Verification items for the finished model (mm, model axes). A direction names the side the tool comes from. Coordinates: 2 decimals unless noted, no trailing zeros. Order: outer loops, then holes, each group sorted by start corner. A loop starts at its lowest first (then second) coordinate and runs counter-clockwise, first axis right, second up.
Q1. Thickness scan on line 1 (Y direction, x = 0.7, z = 1.4); line 2 (X direction, y = 4.9, z = -1.35); line 3 (X direction, y = 2.65, z = 0.5). Record the ranges inside material, lowest first.
Q2. Cross-section at A-A, the plane x = 0. Record the boundary of the cut face in (y, z).
Q3. Cross-section at C-C, the plane y = 3.75. Record the boundary of the cut face in (x, z).
Q4. Cross-section at D-D, the plane y = 2.6. Record the boundary of the cut face in (x, z), and give its area (3 significant figures).
Q5. Cross-section at B-B, the plane z = 0. Record the boundary of the cut face in (x, y), and give its area (3 significant figures).
Q6. Set-up check for faces 1 (the flat face through (0, 0, 0)), 2 (the cylindrical face through (0.45, 1.58, 1.43)): record each of +Z, -Z, +X, -X, +Y, -Y from which the full face is reachable in a straight line by a thin tool's end or side.
Q7. Depth check by flat-ended pin: P1, Ø2, axis at y = 1, z = 1.5, coming from the +X side; P2, Ø1, axis at y = 3.5, z = 1, coming from the -X side. Enter the tip coordinate at first touch or a pass-through.
from build123d import *

# Parameters (mm, degrees)
SKETCH1_R           = 1.5
BOSS_EXTRUDE1_DEPTH = 3
SKETCH2_R           = 2
BOSS_EXTRUDE2_DEPTH = 3
CHAMFER1_SIZE       = 0.2


with BuildPart() as part:
    # Sketch1 → Boss-Extrude1 (new body)
    with BuildSketch(Plane(origin=(0, 0, 0), x_dir=(1, 0, 0), z_dir=(0, 1, 0))):
        with Locations(Location((0, 0, 0), (0, 0, 270))):
            Circle(SKETCH1_R)
    extrude(amount=BOSS_EXTRUDE1_DEPTH)

    # Sketch2 → Boss-Extrude2 (add)
    with BuildSketch(Plane(origin=(0, 3, 0), x_dir=(1, 0, 0), z_dir=(0, 1, 0))):
        with Locations(Location((0, 0, 0), (0, 0, 270))):
            Circle(SKETCH2_R)
    extrude(amount=BOSS_EXTRUDE2_DEPTH)

    # Chamfer1
    chamfer1_edges = [part.edges().sort_by_distance(p)[0] for p in [
        (0, 0, -1.5),
        (0, 6, -2),
    ]]
    chamfer(chamfer1_edges, length=CHAMFER1_SIZE)


solid = part.part
Check values:
1. line 1: y = 3 to 6
1. line 2: x = -1.48 to 1.48
1. line 3: x = -1.41 to 1.41
2. outline: (0, -1.3) - (0.2, -1.5) - (3, -1.5) - (3, -2) - (5.8, -2) - (6, -1.8) - (6, 1.8) - (5.8, 2) - (3, 2) - (3, 1.5) - (0.2, 1.5) - (0, 1.3) - close
3. outline: circle Ø4 at (0, 0)
4. outline: circle Ø3 at (0, 0)
4. area: 7.07 mm2
5. outline: (-2, 3) - (-1.5, 3) - (-1.5, 0.2) - (-1.3, 0) - (1.3, 0) - (1.5, 0.2) - (1.5, 3) - (2, 3) - (2, 5.8) - (1.8, 6) - (-1.8, 6) - (-2, 5.8) - close
5. area: 20.9 mm2
6. face 1: +Z, -Z, +X, -X, -Y
6. face 2: -Y
7. P1: stops at x = 1.41
7. P2: stops at x = -1.94
